Part model, mm, in its own coordinate system. A direction names the side the tool comes from. Coordinates: 2 decimals unless noted, no trailing zeros. Write each loop counter-clockwise with the first axis right and the second up, starting at its lowest first coordinate (ties: lowest second). Pieces come first, ordered by that corner, then holes. Notation, with made-up numbers: (67.5, 42) -> (90.5, 42) arc R17 cw to (90.5, 53) -> close; hole circle Ø2 at (-6, 47.5). An arc over 180 degrees is marked (long way). Write item = value, one per line.
from build123d import *

# Parameters (mm, degrees)
BOSS_EXTRUDE1_DEPTH = 2200
SHELL1_T            = -4
SKETCH2_R           = 3.25
CUT_EXTRUDE1_DEPTH  = 10
CUT_EXTRUDE2_DEPTH  = 2000
SKETCH4_W           = 2035.40419349
SKETCH4_H           = 2143.359963821
CUT_EXTRUDE3_DEPTH  = 2000


with BuildPart() as part:
    # Sketch1 → Boss-Extrude1 (new body)
    with BuildSketch(Plane.XY):
        with BuildLine():
            Line((35, 25), (-35, 25))
            ThreePointArc((-35, 25), (-38.535533906, 23.535533906), (-40, 20))
            Line((-40, 20), (-40, -20))
            ThreePointArc((-40, -20), (-38.535533906, -23.535533906), (-35, -25))
            Line((-35, -25), (35, -25))
            ThreePointArc((35, -25), (38.535533906, -23.535533906), (40, -20))
            Line((40, -20), (40, 20))
            ThreePointArc((40, 20), (38.535533906, 23.535533906), (35, 25))
        make_face()
    extrude(amount=BOSS_EXTRUDE1_DEPTH)

    # Shell1
    shell1_openings = [part.faces().sort_by_distance(p)[0] for p in [
        (0, 0, 2200),
        (0, 0, 0),
    ]]
    offset(amount=SHELL1_T, openings=shell1_openings, kind=Kind.INTERSECTION)

    # Sketch2 → Cut-Extrude1 (cut)
    with BuildSketch(Plane(origin=(0, 25, 0), x_dir=(1, 0, 0), z_dir=(0, 1, 0))):
        with Locations(Location((-25, -919, 0), (0, 0, 180))):
            Circle(SKETCH2_R)
        with Locations(Location((25, -919, 0), (0, 0, 180))):
            Circle(SKETCH2_R)
        with Locations(Location((-25, -849, 0), (0, 0, 180))):
            Circle(SKETCH2_R)
        with Locations(Location((25, -849, 0), (0, 0, 180))):
            Circle(SKETCH2_R)
        with Locations(Location((-25, -1281, 0), (0, 0, 180))):
            Circle(SKETCH2_R)
        with Locations(Location((25, -1281, 0), (0, 0, 180))):
            Circle(SKETCH2_R)
        with Locations(Location((-25, -1351, 0), (0, 0, 180))):
            Circle(SKETCH2_R)
        with Locations(Location((25, -1351, 0), (0, 0, 180))):
            Circle(SKETCH2_R)
    extrude(amount=-CUT_EXTRUDE1_DEPTH, mode=Mode.SUBTRACT)

    # Sketch3 → Cut-Extrude2 (cut)
    with BuildSketch(Plane.XZ.offset(25)):
        Polygon((-40, 2200), (40, 2120), (40, 2200), align=None)
        Polygon((40, 80), (40, 0), (-40, 0), align=None)
    extrude(amount=-CUT_EXTRUDE2_DEPTH, mode=Mode.SUBTRACT)

    # Sketch4 → Cut-Extrude3 (cut)
    with BuildSketch(Plane.XZ.offset(25)):
        with Locations((0, 1191.679981911)):
            Rectangle(SKETCH4_W, SKETCH4_H)
    extrude(amount=-CUT_EXTRUDE3_DEPTH, mode=Mode.SUBTRACT)


solid = part.part
Q1. Saw through at C-C on z = 104. Give the cut face in (x, y).
Model answer:
outline = (-40, -20) arc R5 ccw to (-35, -25) -> (35, -25) arc R5 ccw to (40, -20) -> (40, 20) arc R5 ccw to (35, 25) -> (-35, 25) arc R5 ccw to (-40, 20) -> close; hole (-36, -20) arc R1 ccw to (-35, -21) -> (35, -21) arc R1 ccw to (36, -20) -> (36, 20) arc R1 ccw to (35, 21) -> (-35, 21) arc R1 ccw to (-36, 20) -> close
Q2. Mould opens along Y. For faces 3 (the face through (-7, 21, 74)), 4 (the face through (39, 23, 97)), 5 (the face through (-40, 0, 59)), 6 (the face through (38, -24, 97)) say: released by +Y, released by -Y, zero draft, split by the parting line, or undercut.
Model answer:
face_3 = undercut
face_4 = released by +Y
face_5 = zero draft
face_6 = released by -Y
Q3. Probe line 1 (Y direction, x = -2.5, z = 88); line 2 (X direction, y = -4, z = 106.5); line 3 (X direction, y = -18, z = 14). List the from-to ranges inside material, lowest first. Write a range as from..to.
Model answer:
line_1 = -25..-21, 21..25
line_2 = -40..-36, 36..40
line_3 = -40..-36
Q4. Which spindle directions (+Z, -Z, +X, -X, +Y, -Y) get a long thin tool onto all of the face, cutting with end or side? Do faces 1 (the face through (-38, 24, 59)), 2 (the face through (36, 0, 98)). Say none if no direction does.
Model answer:
face_1 = +Z, -Z, -X, +Y
face_2 = +Z, -Z
Q5. Saw through at B-B on y = 17. Give the cut face in (x, z), and give its area (3 significant figures).
Model answer:
outline = (-40, 0) -> (-36, 4) -> (-36, 120) -> (-40, 120) -> close; (36, 76) -> (40, 80) -> (40, 120) -> (36, 120) -> close
area = 640 mm²
Q6. Saw through at A-A on x = -11. Give the cut face in (y, z), and give its area (3 significant figures).
Model answer:
outline = (-25, 29) -> (-21, 29) -> (-21, 120) -> (-25, 120) -> close; (21, 29) -> (25, 29) -> (25, 120) -> (21, 120) -> close
area = 728 mm²
Q7. Saw through at D-D on z = 68. Give the cut face in (x, y).
Model answer:
outline = (-40, -20) arc R5 ccw to (-35, -25) -> (28, -25) -> (28, -21) -> (-35, -21) arc R1 cw to (-36, -20) -> (-36, 20) arc R1 cw to (-35, 21) -> (28, 21) -> (28, 25) -> (-35, 25) arc R5 ccw to (-40, 20) -> close
Q8. Pin check, flat tips, straight feed: pin 1 (10 mm diameter, centred on x = -7.5, y = 18, fed in from -Z); pin 2 (20 mm diameter, centred on y = 5, z = 65.5, fed in from +X); pin 3 (8 mm diameter, centred on y = 18.5, z = 78.5, fed in from +X). Stop position of each tip, or through.
Model answer:
pin_1 = 28.5
pin_2 = -36
pin_3 = 40
